```python
from build123d import *

# Parameters (mm, degrees)
SKETCH_1_W                   = 100
SKETCH_1_H                   = 106
EXTRUDE_1_DEPTH              = 5
HOLE_WIZARD_M5_1_D           = 4.2
CHAMFER_1_SIZE               = 8
HOLE_WIZARD_M4_1_D           = 3.3
SKETCH_10_R                  = 6
EXTRUDE1_DEPTH               = 74.545904033
M3_TAPPED_HOLE1_D            = 2.5
SKETCH3_R                    = 14.5
EXTRUDE2_DEPTH               = 5
F_8_0_8_DIAMETER_HOLE1_D     = 8
F_8_0_8_DIAMETER_HOLE1_DEPTH = 24
F_8_0_8_DIAMETER_HOLE1_TIP   = 2.403442476
SKETCH6_R                    = 6.5
EXTRUDE3_DEPTH               = 5


with BuildPart() as part:
    # 草图1 → 凸台-拉伸1 (new, symmetric)
    with BuildSketch(Plane.XY):
        Rectangle(SKETCH_1_W, SKETCH_1_H)
    extrude(amount=EXTRUDE_1_DEPTH, both=True)

    # M5 螺纹孔1 (through all)
    with Locations(Plane.XY.offset(5)):
        with Locations((-35, 0), (35, 0)):
            Hole(HOLE_WIZARD_M5_1_D / 2)

    # 倒角1
    chamfer_1_edges = [part.edges().sort_by_distance(p)[0] for p in [
        (50, -53, 0),
        (-50, -53, 0),
        (-50, 53, 0),
        (50, 53, 0),
    ]]
    chamfer(chamfer_1_edges, length=CHAMFER_1_SIZE)

    # M4 螺纹孔1 (through all)
    with Locations(Plane.XY.offset(5)):
        with Locations((-40, -7.5), (-40, 7.5)):
            hole_wizard_m4_1 = Hole(HOLE_WIZARD_M4_1_D / 2)

    # 镜向2: M4 螺纹孔1 across plane
    add(hole_wizard_m4_1.mirror(Plane(origin=(0, 0, 0), x_dir=(0, 0, 1), z_dir=(1, 0, 0))), mode=Mode.SUBTRACT)

    # 草图10 → Extrude1 (cut, through all)
    with BuildSketch(Plane.XY.offset(5)):
        with Locations((-20, 42.5)):
            Circle(SKETCH_10_R)
        with Locations((-20, -42.5)):
            Circle(SKETCH_10_R)
        with Locations((20, -42.5)):
            Circle(SKETCH_10_R)
        with Locations((20, 42.5)):
            Circle(SKETCH_10_R)
    extrude(amount=-EXTRUDE1_DEPTH, mode=Mode.SUBTRACT)

    # M3 Tapped Hole1 (through all)
    with Locations(Plane.XY.offset(5)):
        with Locations((10, -42.5), (30, -42.5), (-10, -42.5), (-30, -42.5), (-10, 42.5), (-30, 42.5), (10, 42.5), (30, 42.5)):
            Hole(M3_TAPPED_HOLE1_D / 2)

    # Sketch3 → Extrude2 (cut)
    with BuildSketch(Plane.XY.offset(-5)):
        with Locations((-20, 42.5)):
            Circle(SKETCH3_R)
        with Locations((-20, -42.5)):
            Circle(SKETCH3_R)
        with Locations((20, -42.5)):
            Circle(SKETCH3_R)
        with Locations((20, 42.5)):
            Circle(SKETCH3_R)
    extrude(amount=EXTRUDE2_DEPTH, mode=Mode.SUBTRACT)

    # Ø8.0 (8) Diameter Hole1
    with Locations(Plane.XY.offset(5)):
        with Locations((-42, 42.5), (42, 42.5), (42, -42.5), (-42, -42.5)):
            Hole(F_8_0_8_DIAMETER_HOLE1_D / 2, depth=F_8_0_8_DIAMETER_HOLE1_DEPTH)
            with Locations((0, 0, -(F_8_0_8_DIAMETER_HOLE1_DEPTH + F_8_0_8_DIAMETER_HOLE1_TIP / 2))):  # 118° drill point
                Cone(0, F_8_0_8_DIAMETER_HOLE1_D / 2, F_8_0_8_DIAMETER_HOLE1_TIP, mode=Mode.SUBTRACT)

    # Sketch6 → Extrude3 (cut)
    with BuildSketch(Plane(origin=(0, 0, -5), x_dir=(-1, 0, 0), z_dir=(0, 0, -1))):
        with Locations((42, -42.5)):
            Circle(SKETCH6_R)
        with Locations((-42, -42.5)):
            Circle(SKETCH6_R)
        with Locations((42, 42.5)):
            Circle(SKETCH6_R)
        with Locations((-42, 42.5)):
            Circle(SKETCH6_R)
    extrude(amount=-EXTRUDE3_DEPTH, mode=Mode.SUBTRACT)


solid = part.part
```
Can you work these out from the model? Positions are in its coordinate system, mm. A direction names the side the tool comes from. Round coordinates to 2 decimals unless told otherwise and drop trailing zeros. Order: outer loops, then holes, each group sorted by start corner. A loop starts at its lowest first (then second) coordinate and runs counter-clockwise, first axis right, second up.
(1) On a 3-axis mill with a long thin cutter (end or side, diameter ignored), from which of +Z, -Z, +X, -X, +Y, -Y can I reach the whole of each face in a straight line? I mean faces 5 (the face through (-14, 41, 0)), 6 (the face through (25.54, 40.2, 2.54)). Say none if no direction works.
Results are:
face 5: -Z
face 6: +Z, -Z
(2) I'm going to push flat-ended pins straight in: pin 1 (7 mm diameter, centred on x = 20, y = 42.5, fed in from +Z); pin 2 (19 mm diameter, centred on x = 20, y = -42.5, fed in from -Z); pin 3 (3 mm diameter, centred on x = 22, z = -2.5, fed in from -Y). Where does each tip first touch, or does it pass through?
Results are:
pin 1: passes through
pin 2: stops at z = 0
pin 3: stops at y = -28.43
(3) If we section it at A-A (z = 3.75): Count the separate pieces of the cut face and the enclosed holes in it, plus the area to 3 significant figures.
Results are:
separate pieces: 1
enclosed holes: 22
area: 9,720 mm2
(4) If we section it at B-B (x = -23.5): Please give me the cut outline in (y, z), plus the area to 3 significant figures.
Results are:
outline: (-53, 0) - (-47.37, 0) - (-47.37, 5) - (-53, 5) - close; (-37.63, 0) - (-28.43, 0) - (-28.43, -5) - (28.43, -5) - (28.43, 0) - (37.63, 0) - (37.63, 5) - (-37.63, 5) - close; (47.37, 0) - (53, 0) - (53, 5) - (47.37, 5) - close
area: 717 mm2
(5) If we section it at D-D (y = 29.5): Please give me the cut outline in (x, z).
Results are:
outline: (-50, -5) - (-26.42, -5) - (-26.42, 0) - (-13.58, 0) - (-13.58, -5) - (13.58, -5) - (13.58, 0) - (26.42, 0) - (26.42, -5) - (50, -5) - (50, 5) - (-50, 5) - close
(6) If I drill on L1, parallel to Y at x = 10, z = 1.8; L2, parallel to Y at x = -42, z = -1.7; L3, parallel to X at y = -38, z = 0.5, over which ranges is the centre line in solid material (lowest first)?
Results are:
L1: y = -53 to -43.75, -41.25 to 41.25, 43.75 to 53
L2: y = -53 to -49, -36 to 36, 49 to 53
L3: x = -50 to -23.97, -16.03 to 16.03, 23.97 to 50
(7) We'd pull the mould along Y, two halves only. Please class faces 1 (the face through (46, -49, 0)), 2 (the face through (-9.84, 43.74, 2.47)), 3 (the face through (-1, 53, 1)), 4 (the face through (-20, -28, -3)): +Y half, -Y half, draft (parallel to the pull), parting line (faces both ways), or undercut.
Results are:
face 1: -Y half
face 2: undercut
face 3: +Y half
face 4: undercut
